```python
from build123d import *

# Parameters (mm, degrees)
SKETCH1_R           = 17.5
BOSS_EXTRUDE1_DEPTH = 2
SKETCH3_R           = 4
BOSS_EXTRUDE2_DEPTH = 2
CHAMFER1_SIZE       = 1
SKETCH4_R           = 2
BOSS_EXTRUDE3_DEPTH = 15
SKETCH5_R           = 1.5
CUT_EXTRUDE1_DEPTH  = 15
SKETCH6_R           = 1
BOSS_EXTRUDE4_DEPTH = 8
SKETCH7_W           = 4
SKETCH7_H           = 45.60719986
CUT_EXTRUDE2_DEPTH  = 32.200961524
SKETCH8_R           = 2
CUT_EXTRUDE3_DEPTH  = 3


with BuildPart() as part:
    # Sketch1 → Boss-Extrude1 (new body)
    with BuildSketch(Plane(origin=(0, 0, 0), x_dir=(1, 0, 0), z_dir=(0, 1, 0))):
        with Locations(Location((0, 0, 0), (0, 0, 270))):
            Circle(SKETCH1_R)
    extrude(amount=BOSS_EXTRUDE1_DEPTH)

    # Sketch3 → Boss-Extrude2 (add)
    with BuildSketch(Plane.XZ):
        with Locations(Location((0, 0, 0), (0, 0, 270))):
            Circle(SKETCH3_R)
    extrude(amount=BOSS_EXTRUDE2_DEPTH)

    # Chamfer1
    chamfer1_edges = [part.edges().sort_by_distance(p)[0] for p in [
        (0, 0, 4),
    ]]
    chamfer(chamfer1_edges, length=CHAMFER1_SIZE)

    # Sketch4 → Boss-Extrude3 (add)
    with BuildSketch(Plane.XZ.offset(2)):
        with Locations(Location((0, 0, 0), (0, 0, 270))):
            Circle(SKETCH4_R)
    extrude(amount=BOSS_EXTRUDE3_DEPTH)

    # Sketch5 → Cut-Extrude1 (cut)
    with BuildSketch(Plane.XZ.offset(17)):
        with Locations(Location((0, 0, 0), (0, 0, 270))):
            Circle(SKETCH5_R)
    extrude(amount=-CUT_EXTRUDE1_DEPTH, mode=Mode.SUBTRACT)

    # Sketch6 → Boss-Extrude4 (add)
    with BuildSketch(Plane(origin=(0, 2, 0), x_dir=(1, 0, 0), z_dir=(0, 1, 0))):
        with Locations(Location((-10, 0, 0), (0, 0, 270))):
            Circle(SKETCH6_R)
        with Locations(Location((8.838834765, 8.838834765, 0), (0, 0, 270))):
            Circle(SKETCH6_R)
    extrude(amount=BOSS_EXTRUDE4_DEPTH)

    # Sketch7 → Cut-Extrude2 (cut, through all)
    with BuildSketch(Plane(origin=(0, 2, 0), x_dir=(1, 0, 0), z_dir=(0, 1, 0))):
        with Locations((-15.5, 0)):
            Rectangle(SKETCH7_W, SKETCH7_H)
    extrude(amount=-CUT_EXTRUDE2_DEPTH, mode=Mode.SUBTRACT)

    # Sketch8 → Cut-Extrude3 (cut)
    with BuildSketch(Plane(origin=(0, 2, 0), x_dir=(1, 0, 0), z_dir=(0, 1, 0))):
        with Locations(Location((0, 0, 0), (0, 0, 90))):
            Circle(SKETCH8_R)
    extrude(amount=-CUT_EXTRUDE3_DEPTH, mode=Mode.SUBTRACT)


solid = part.part
```
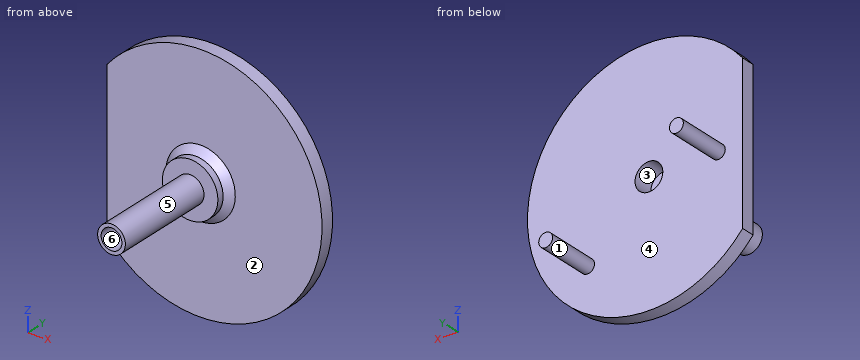
Source: CAD feature listing. Evaluate the final solid. Frame: model axes, mm. Face numbers are marked on the shaded views. A direction names the side the tool comes from. Coordinates: 2 decimals unless noted, no trailing zeros. Write each loop counter-clockwise with the first axis right and the second up, starting at its lowest first coordinate (ties: lowest second). Pieces come first, ordered by that corner, then holes. Notation, with made-up numbers: (30.25, -1) -> (89.25, -1) arc R8 ccw to (89.25, 8) -> close; hole circle Ø1 at (1.25, 38.25). An arc over 180 degrees is marked (long way). Return JSON: item names as keys, results as strings. Group by question number.
1) Mould query, pull axis Z, two halves, no side actions, for the marked faces 3, 4, 5 and 6. Classes: +Z half, -Z half, draft (parallel to the pull), parting line (faces both ways), or undercut.
2) Set-up query: the marked faces 1 and 2. Return all of +Z, -Z, +X, -X, +Y, -Y with unobstructed straight access to the full face (end or side cutting, diameter ignored); none if empty.
3) Section query D-D, the plane y = 7.5. Return loops of the section in (x, z).
4) Section query B-B, the plane x = 0. Return loops of the section in (y, z).
5) Section query A-A, the plane z = 0. Return loops of the section in (x, y).
6) Contact query for flat-ended pins moving along their axis: P1, Ø4.5, axis at x = 0, z = 0, coming from the -Y side; P2, Ø10, axis at x = 12, z = -1, coming from the -Y side; P3, Ø2, axis at y = -4, z = 0.5, coming from the -X side; P4, Ø5, axis at y = 0, z = -4, coming from the +X side. Output: stop coordinate, or through.
7) Section query C-C, the plane y = -11. Return loops of the section in (x, z).
8) Ray query, line 1 along X through (y, z) = (0.55, 0); line 2 along X through (y, z) = (-4.5, 0); line 3 along Y through (x, z) = (-10, -13). Return the intervals inside material, ascending.
From the geometry:
{
 "1": {"face 3": "undercut", "face 4": "draft", "face 5": "parting line", "face 6": "undercut"},
 "2": {"face 1": "+Y", "face 2": "-Y"},
 "3": {"outline": "circle Ø2 at (-10, 0); circle Ø2 at (8.84, -8.84)"},
 "4": {"outline": "(-17, -2) -> (-2, -2) -> (-2, -4) -> (-1, -4) -> (0, -5) -> (0, -17.5) -> (2, -17.5) -> (2, -2) -> (-1, -2) -> (-1, 2) -> (2, 2) -> (2, 17.5) -> (0, 17.5) -> (0, 5) -> (-1, 4) -> (-2, 4) -> (-2, 2) -> (-17, 2) -> (-17, 1.5) -> (-2, 1.5) -> (-2, -1.5) -> (-17, -1.5) -> close"},
 "5": {"outline": "(-13.5, 0) -> (-5, 0) -> (-4, -1) -> (-4, -2) -> (-2, -2) -> (-2, -17) -> (-1.5, -17) -> (-1.5, -2) -> (1.5, -2) -> (1.5, -17) -> (2, -17) -> (2, -2) -> (4, -2) -> (4, -1) -> (5, 0) -> (17.5, 0) -> (17.5, 2) -> (2, 2) -> (2, -1) -> (-2, -1) -> (-2, 2) -> (-9, 2) -> (-9, 10) -> (-11, 10) -> (-11, 2) -> (-13.5, 2) -> close"},
 "6": {"P1": "y = -17", "P2": "y = 0", "P3": "x = -2", "P4": "x = 17.44"},
 "7": {"outline": "circle Ø4 at (0, 0); hole circle Ø3 at (0, 0)"},
 "8": {"line 1": "-13.5 to -2, 2 to 17.5", "line 2": "-2 to -1.5, 1.5 to 2", "line 3": "0 to 2"}
}
